```python
from build123d import *
from OCP.BRepFilletAPI import BRepFilletAPI_MakeChamfer

# Parameters (mm, degrees)
BOSS_EXTRUDE1_DEPTH        = 40
CHAMFER1_SIZE              = 3
CHAMFER2_SIZE              = 1
CHAMFER2_SIZE2             = 0.96684652
CHAMFER2_SIZE2_2           = 1.036815955
CHAMFER2_SIZE2_3           = 0.976206784
CHAMFER2_SIZE2_4           = 1.025622313
HOLE2_D                    = 6.6
HOLE2_DEPTH                = 20
SKETCH11_W                 = 5.5
SKETCH11_H                 = 19.966257543
HOLE3_AT_2_COUNT           = 2
HOLE3_AT_2_PITCH           = 46.626722383
SIZE_MM_BLIND_HOLE_1_D     = 8
SIZE_MM_BLIND_HOLE_1_DEPTH = 12.5
SIZE_MM_BLIND_HOLE_1_TIP   = 2.403442476


with BuildPart() as part:
    # Sketch2 → Boss-Extrude1 (new body)
    with BuildSketch(Plane.XY):
        Polygon((-37.58146769, 20.630053858), (22.41853231, 22.725300027), (22.41853231, 60.630053858), (-37.58146769, 60.630053858), align=None)
    extrude(amount=BOSS_EXTRUDE1_DEPTH)

    # Chamfer1
    chamfer1_edges = [part.edges().sort_by_distance(p)[0] for p in [
        (22.41853231, 41.677676942, 40),
        (-37.58146769, 40.630053858, 40),
        (22.41853231, 41.677676942, 0),
        (-37.58146769, 40.630053858, 0),
    ]]
    chamfer(chamfer1_edges, length=CHAMFER1_SIZE)

    # Chamfer2: one chamfer whose edges measure the first distance from different faces: ONE call of the kernel's chamfer builder (chamfer() names one face for all edges)
    chamfer2_edges_1 = [part.edges().sort_by_distance(p)[0] for p in [
        (-37.58146769, 20.630053858, 20),
    ]]
    chamfer2_side_1 = [part.faces().sort_by_distance(p)[0] for p in [
        (-37.58146769, 40.630053858, 20),
    ]]
    chamfer2_edges_2 = [part.edges().sort_by_distance(p)[0] for p in [
        (-7.58146769, 21.677676942, 0),
        (-7.58146769, 21.677676942, 40),
    ]]
    chamfer2_edges_3 = [part.edges().sort_by_distance(p)[0] for p in [
        (22.41853231, 22.725300027, 20),
    ]]
    chamfer2_side_3 = [part.faces().sort_by_distance(p)[0] for p in [
        (-7.58146769, 21.677676942, 20),
    ]]
    chamfer2_edges_4 = [part.edges().sort_by_distance(p)[0] for p in [
        (-36.08146769, 20.682435012, 38.5),
    ]]
    chamfer2_side_4 = [part.faces().sort_by_distance(p)[0] for p in [
        (-36.082123313, 40.656232987, 38.499344377),
    ]]
    chamfer2_edges_5 = [part.edges().sort_by_distance(p)[0] for p in [
        (20.91853231, 22.672918873, 38.5),
    ]]
    chamfer2_side_5 = [part.faces().sort_by_distance(p)[0] for p in [
        (20.917842306, 41.651474317, 38.500690004),
    ]]
    chamfer2_edges_6 = [part.edges().sort_by_distance(p)[0] for p in [
        (20.91853231, 22.672918873, 1.5),
    ]]
    chamfer2_side_6 = [part.faces().sort_by_distance(p)[0] for p in [
        (20.917842306, 41.651474317, 1.499309996),
    ]]
    chamfer2_edges_7 = [part.edges().sort_by_distance(p)[0] for p in [
        (-36.08146769, 20.682435012, 1.5),
    ]]
    chamfer2_side_7 = [part.faces().sort_by_distance(p)[0] for p in [
        (-36.082123313, 40.656232987, 1.500655623),
    ]]
    chamfer2 = BRepFilletAPI_MakeChamfer(part.part.solid().wrapped)
    for e in chamfer2_edges_1:
        chamfer2.Add(CHAMFER2_SIZE, CHAMFER2_SIZE2, e.wrapped, chamfer2_side_1[0].wrapped)  # the first distance lies on this face
    for e in chamfer2_edges_2:
        chamfer2.Add(CHAMFER2_SIZE, e.wrapped)
    for e in chamfer2_edges_3:
        chamfer2.Add(CHAMFER2_SIZE, CHAMFER2_SIZE2_2, e.wrapped, chamfer2_side_3[0].wrapped)  # the first distance lies on this face
    for e in chamfer2_edges_4:
        chamfer2.Add(CHAMFER2_SIZE, CHAMFER2_SIZE2_3, e.wrapped, chamfer2_side_4[0].wrapped)  # the first distance lies on this face
    for e in chamfer2_edges_5:
        chamfer2.Add(CHAMFER2_SIZE, CHAMFER2_SIZE2_4, e.wrapped, chamfer2_side_5[0].wrapped)  # the first distance lies on this face
    for e in chamfer2_edges_6:
        chamfer2.Add(CHAMFER2_SIZE, CHAMFER2_SIZE2_4, e.wrapped, chamfer2_side_6[0].wrapped)  # the first distance lies on this face
    for e in chamfer2_edges_7:
        chamfer2.Add(CHAMFER2_SIZE, CHAMFER2_SIZE2_3, e.wrapped, chamfer2_side_7[0].wrapped)  # the first distance lies on this face
    add(Compound.cast(chamfer2.Shape()), mode=Mode.REPLACE)

    # Hole2
    with Locations(Plane(origin=(0, 60.630053858, 0), x_dir=(1, 0, 0), z_dir=(0, 1, 0))):
        with Locations((-27.514846728, -32), (12.460786352, -8)):
            Hole(HOLE2_D / 2, depth=HOLE2_DEPTH)

    # Sketch11 → Hole3 (revolve, cut)
    with BuildSketch(Plane(origin=(-27.514846728, 40.630053858, 32), x_dir=(0, 0, 1), z_dir=(1, 0, 0))):
        with Locations((2.75, 9.983128772)):
            Rectangle(SKETCH11_W, SKETCH11_H)
    hole3 = revolve(axis=Axis((-27.514846728, -69.369946142, 32), (0, 1, 0)), mode=Mode.SUBTRACT)

    # Hole3 at 2: Hole3 ×2
    with Locations(*[Vector(0.8573545605919571, 0, -0.514726293705861) * (i * HOLE3_AT_2_PITCH) for i in range(1, HOLE3_AT_2_COUNT)]):
        add(hole3, mode=Mode.SUBTRACT)

    # Size mm blind hole 1
    with Locations(Plane(origin=(0, 60.630053858, 0), x_dir=(1, 0, 0), z_dir=(0, 1, 0))):
        with Locations((-27.514846728, -8), (12.460786352, -32)):
            Hole(SIZE_MM_BLIND_HOLE_1_D / 2, depth=SIZE_MM_BLIND_HOLE_1_DEPTH)
            with Locations((0, 0, -(SIZE_MM_BLIND_HOLE_1_DEPTH + SIZE_MM_BLIND_HOLE_1_TIP / 2))):  # 118° drill point
                Cone(0, SIZE_MM_BLIND_HOLE_1_D / 2, SIZE_MM_BLIND_HOLE_1_TIP, mode=Mode.SUBTRACT)


solid = part.part
```
Verification items for the finished model (mm, model axes). A direction names the side the tool comes from. Round coordinates to 2 decimals unless told otherwise and drop trailing zeros. Write each loop counter-clockwise with the first axis right and the second up, starting at its lowest first coordinate (ties: lowest second). Pieces come first, ordered by that corner, then holes. Notation, with made-up numbers: (35.5, 0) - (42.5, 0) arc R23 ccw to (42.5, 10) - close; hole circle Ø2 at (71.25, 10). An arc over 180 degrees is marked (long way). Answer as a JSON object with one key per item and string values. Group by question number.
Q1. Section check C-C, the plane x = -19. Enter the section's corners in (y, z), plus the area to 3 significant figures.
Q2. Mould release check, pull along X, two halves, no side actions. Record for faces 1 (the flat face through (-36.06, 41.4, 1.48)), 2 (the flat face through (-8, 41, 40)), 3 (the flat face through (-27, 40.63, 28)): released by +X, released by -X, zero draft, split by the parting line, or undercut.
Q3. Thickness scan on line 1 (X direction, y = 51.25, z = 32); line 2 (X direction, y = 50, z = 9); line 3 (Z direction, x = 11, y = 28.5). Record the ranges inside material, lowest first.
Q4. Section check B-B, the plane y = 32.5. Enter the section's corners in (x, z), plus the area to 3 significant figures.
Q5. Tool access check on faces 4 (the flat face through (-8, 41, 0)), 5 (the flat face through (13, 40.63, 4)), 6 (the cylindrical face through (-24.34, 54.29, 10.43)). Record the directions out of +Z, -Z, +X, -X, +Y, -Y that give a thin tool (end or side, any length) a straight path to the whole face; none if there is none.
Q6. Go/stop test with flat-tipped pins: pin 1 Ø6.5 at (x, z) = (-27.51, 8) entering from -Y; pin 2 Ø17.5 at (x, z) = (-27.51, 32) entering from -Y; pin 3 Ø12 at (x, z) = (9.5, 9) entering from -Y. Record where each tip stops, or that it passes through.
Q7. Section check A-A, the plane z = 23. Enter the section's corners in (x, y).
Found:
{
 "1": {"outline": "(21.28, 1) - (22.28, 0) - (60.63, 0) - (60.63, 40) - (22.28, 40) - (21.28, 39) - close", "area": "1,570 mm^2"},
 "2": {"face 1": "released by -X", "face 2": "zero draft", "face 3": "undercut"},
 "3": {"line 1": "x = -37.58 to -30.81, -24.21 to 8.46, 16.46 to 22.42", "line 2": "x = -37.58 to -31.39, -23.64 to 9.32, 15.61 to 22.42", "line 3": "z = 0 to 2.7, 13.3 to 40"},
 "4": {"outline": "(-37.58, 3) - (-34.58, 0) - (19.42, 0) - (22.42, 3) - (22.42, 37) - (19.42, 40) - (-34.58, 40) - (-37.58, 37) - close; hole circle Ø11 at (-27.51, 32); hole circle Ø11 at (12.46, 8)", "area": "2,190 mm^2"},
 "5": {"face 4": "-Z, +X, -X, +Y, -Y", "face 5": "-Y", "face 6": "+Y"},
 "6": {"pin 1": "stops at y = 20.87", "pin 2": "stops at y = 20.68", "pin 3": "stops at y = 22.06"},
 "7": {"outline": "(-37.58, 21.63) - (-36.62, 20.66) - (21.42, 22.69) - (22.42, 23.76) - (22.42, 60.63) - (-37.58, 60.63) - close"}
}
